Can you work these out from the model? Positions are in its coordinate system, mm. Give positions to 0.01 mm unless a question says otherwise; leave off trailing zeros. Write each loop counter-clockwise with the first axis right and the second up, starting at its lowest first coordinate (ties: lowest second). Pieces come first, ordered by that corner, then holes.
from build123d import *

# Parameters (mm, degrees)
BOSS_EXTRUDE1_DEPTH                         = 5
HOLE_SIZE_BY_HEX_SOCKET_COUNTERSUNK_2_COUNT = 2
HOLE_SIZE_BY_HEX_SOCKET_COUNTERSUNK_2_PITCH = 40


with BuildPart() as part:
    # Sketch1 → Boss-Extrude1 (new body)
    with BuildSketch(Plane(origin=(0, 0, 0), x_dir=(0, 0, -1), z_dir=(1, 0, 0))):
        with BuildLine():
            Line((-45, 60), (-45, 0))
            Line((-45, 0), (45, 0))
            Line((45, 0), (45, 60))
            ThreePointArc((45, 60), (43.535533906, 63.535533906), (40, 65))
            Line((40, 65), (-40, 65))
            ThreePointArc((-40, 65), (-43.535533906, 63.535533906), (-45, 60))
        make_face()
    extrude(amount=BOSS_EXTRUDE1_DEPTH)

    # Sketch2 → Hole size by hex socket countersunk screw type1 (revolve, cut)
    with BuildSketch(Plane(origin=(0, 45, -20), x_dir=(0, 0, 1), z_dir=(0, 1, 0))):
        Polygon((0, 0), (0, 5), (3.3, 5), (3.3, 3.1), (6.4, 0), align=None)
    hole_size_by_hex_socket_countersunk_scre = revolve(axis=Axis((-6.35, 45, -20), (1, 0, 0)), mode=Mode.SUBTRACT)

    # Hole size by hex socket countersunk  2: Hole size by hex socket countersunk screw type1 ×2
    with Locations(*[(0, 0, i * HOLE_SIZE_BY_HEX_SOCKET_COUNTERSUNK_2_PITCH) for i in range(1, HOLE_SIZE_BY_HEX_SOCKET_COUNTERSUNK_2_COUNT)]):
        add(hole_size_by_hex_socket_countersunk_scre, mode=Mode.SUBTRACT)


solid = part.part
(1) Imagine slicing it at C-C, the plane x = 1.3. Write out the boundary of the cut face in (y, z).
Returned:
outline: (0, -45) - (60, -45) arc R5 ccw to (65, -40) - (65, 40) arc R5 ccw to (60, 45) - (0, 45) - close; hole circle Ø10.2 at (45, -20); hole circle Ø10.2 at (45, 20)
(2) If we mould it in two halves opening along Y, with no side actions, what happens to faces 1 (the face through (2, 63, -44)), 2 (the face through (2, 30, 45)), 3 (the face through (4.04, 41.73, -20.43))? For each: +Y half, -Y half, draft (parallel to the pull), parting line (faces both ways), or undercut.
Returned:
face 1: +Y half
face 2: draft
face 3: undercut
(3) Imagine slicing it at A-A, the plane z = 20. Write out the boundary of the cut face in (x, y), plus the area to 3 significant figures.
Returned:
outline: (0, 0) - (5, 0) - (5, 41.7) - (3.1, 41.7) - (0, 38.6) - close; (0, 51.4) - (3.1, 48.3) - (5, 48.3) - (5, 65) - (0, 65) - close
area: 282 mm2
(4) Will these pins go through, and if not, where does the flat tip stop? P1, Ø8.5, axis at y = 45, z = -20, coming from the -X side; P2, Ø10.5, axis at y = 45, z = 20, coming from the -X side.
Returned:
P1: stops at x = 2.15
P2: stops at x = 1.15
(5) If I drill on L1, parallel to Z at x = 3.7, y = 45; L2, parallel to Y at x = 4.6, z = 20; L3, parallel to Y at x = 0.55, z = -17, over which ranges is the centre line in solid material (lowest first)?
Returned:
L1: z = -45 to -23.3, -16.7 to 16.7, 23.3 to 45
L2: y = 0 to 41.7, 48.3 to 65
L3: y = 0 to 39.98, 50.02 to 65
(6) Imagine slicing it at B-B, the plane y = 45. Write out the boundary of the cut face in (x, z).
Returned:
outline: (0, -45) - (5, -45) - (5, -23.3) - (3.1, -23.3) - (0, -26.4) - close; (0, -13.6) - (3.1, -16.7) - (5, -16.7) - (5, 16.7) - (3.1, 16.7) - (0, 13.6) - close; (0, 26.4) - (3.1, 23.3) - (5, 23.3) - (5, 45) - (0, 45) - close
